Source: CAD feature listing. Evaluate the final solid. Frame: model axes, mm. Face numbers are marked on the shaded views. A direction names the side the tool comes from. Coordinates: 2 decimals unless noted, no trailing zeros. Write each loop counter-clockwise with the first axis right and the second up, starting at its lowest first coordinate (ties: lowest second). Pieces come first, ordered by that corner, then holes. Notation, with made-up numbers: (-6, -16) -> (27, -16) arc R21 cw to (27, 7) -> close; hole circle Ø5 at (49.5, 7.25). An arc over 180 degrees is marked (long way). One line per item, written item: value. Start each with the question number.
1. Section query A-A, the plane y = 0. Output: boundary loops of the cut face in (x, z), and give its area (3 significant figures).
2. Section query B-B, the plane x = 0. Output: boundary loops of the cut face in (y, z), and give its area (4 significant figures).
3. Access query for the marked faces 1, 2, 3, 4 and 5. Directions: +Z, -Z, +X, -X, +Y, -Y. A direction counts if a zero-diameter tool reaches every point of the face in a straight line with its end or side. Return the directions, or none.
4. Line query: line 1 (Z direction, x = 38, y = 0); line 2 (Y direction, x = 58, z = 7); line 3 (Z direction, x = -39, y = -37). Output: solid intervals per line, ascending.
5. First-contact query: P1, Ø8, axis at x = -40.5, y = 37.5, coming from the -Z side; P2, Ø5, axis at x = 61.5, z = 11, coming from the -Y side; P3, Ø3, axis at y = -37, z = 7.5, coming from the +X side; P4, Ø1, axis at x = -9, y = -33, coming from the +Z side. Flat tips, straight axial feed; report the tip coordinate or a pass-through.
from build123d import *

# Parameters (mm, degrees)
SKETCH_1_R      = 62
EXTRUDE_1_DEPTH = 4
SKETCH_2_R      = 52
EXTRUDE_2_DEPTH = 4
EXTRUDE_3_DEPTH = 9.5
FILLET_1_R      = 5
CHAMFER_1_SIZE  = 0.5


with BuildPart() as part:
    # 草图1 → 凸台-拉伸1 (new body)
    with BuildSketch(Plane.XY):
        Circle(SKETCH_1_R)
    extrude(amount=EXTRUDE_1_DEPTH)

    # 草图2 → 凸台-拉伸2 (add)
    with BuildSketch(Plane.XY.offset(4)):
        Circle(SKETCH_2_R)
    extrude(amount=EXTRUDE_2_DEPTH)

    # 草图3 → 凸台-拉伸3 (add, symmetric)
    with BuildSketch(Plane(origin=(0, 0, 0), x_dir=(1, 0, 0), z_dir=(0, 1, 0))):
        with BuildLine():
            Line((81, 0), (81, -11.5))
            ThreePointArc((81, -11.5), (79.535533906, -15.035533906), (76, -16.5))
            Line((76, -16.5), (63.5, -16.5))
            Line((63.5, -16.5), (47, -8))
            Line((47, -8), (47, 0))
            Line((47, 0), (81, 0))
        make_face()
        with BuildLine():
            Line((73.5, -5), (73.5, -7.5))
            ThreePointArc((73.5, -7.5), (73.207106781, -8.207106781), (72.5, -8.5))
            Line((72.5, -8.5), (65, -8.5))
            ThreePointArc((65, -8.5), (62.5, -11), (65, -13.5))
            Line((65, -13.5), (72.5, -13.5))
            ThreePointArc((72.5, -13.5), (76.742640687, -11.742640687), (78.5, -7.5))
            Line((78.5, -7.5), (78.5, -5))
            ThreePointArc((78.5, -5), (76, -2.5), (73.5, -5))
        make_face(mode=Mode.SUBTRACT)
    extrude(amount=EXTRUDE_3_DEPTH, both=True)

    # 圆角1
    fillet_1_edges = [part.edges().sort_by_distance(p)[0] for p in [
        (81, 0, 0),
    ]]
    fillet(fillet_1_edges, radius=FILLET_1_R)

    # 倒角1
    chamfer_1_edges = [part.edges().sort_by_distance(p)[0] for p in [
        (-62, 0, 4),
        (-52, 0, 8),
    ]]
    chamfer(chamfer_1_edges, length=CHAMFER_1_SIZE)


solid = part.part
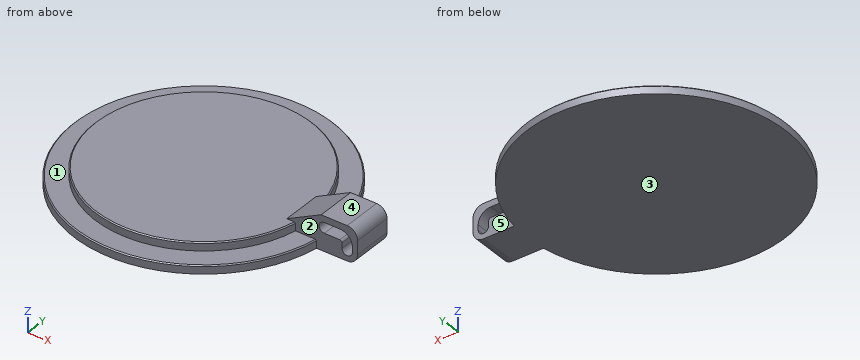
Computed values:
1. outline: (-62, 0) -> (76, 0) arc R5 ccw to (81, 5) -> (81, 11.5) arc R5 ccw to (76, 16.5) -> (63.5, 16.5) -> (47, 8) -> (-51.5, 8) -> (-52, 7.5) -> (-52, 4) -> (-61.5, 4) -> (-62, 3.5) -> close; hole (65, 8.5) -> (72.5, 8.5) arc R1 cw to (73.5, 7.5) -> (73.5, 5) arc R2.5 ccw to (78.5, 5) -> (78.5, 7.5) arc R6 ccw to (72.5, 13.5) -> (65, 13.5) arc R2.5 ccw to start
1. area: 1,210 mm²
2. outline: (-62, 0) -> (62, 0) -> (62, 3.5) -> (61.5, 4) -> (52, 4) -> (52, 7.5) -> (51.5, 8) -> (-51.5, 8) -> (-52, 7.5) -> (-52, 4) -> (-61.5, 4) -> (-62, 3.5) -> close
2. area: 911.5 mm²
3. face 1: +Z
3. face 2: +Z, +X, -Y
3. face 3: -Z, +X, -X, +Y, -Y
3. face 4: +Z, +X, -X, +Y, -Y
3. face 5: +Z, +X, +Y
4. line 1: z = 0 to 8
4. line 2: y = -9.5 to 9.5
4. line 3: z = 0 to 4
5. P1: stops at z = 0
5. P2: stops at y = -9.5
5. P3: stops at x = 38
5. P4: stops at z = 8
